Check sheet for the modelled part. Datum: model origin and axes. Units: mm. Face numbers are marked on the shaded views. Round coordinates to 2 decimals unless told otherwise and drop trailing zeros. Order: outer loops, then holes, each group sorted by start corner. A loop starts at its lowest first (then second) coordinate and runs counter-clockwise, first axis right, second up. Notation, with made-up numbers: (54.25, 58.25) -> (112.25, 58.25) arc R9 cw to (112.25, 69.25) -> close; hole circle Ø10 at (52.5, 29). An arc over 180 degrees is marked (long way). Answer in a Markdown table with one row per item.
from build123d import *

# Parameters (mm, degrees)
EXTRUDE_1_DEPTH             = 1.5
SKETCH_2_W                  = 12.5
SKETCH_2_H                  = 13.5
HOLE_WIZARD_12_0_12_1_D     = 12
HOLE_WIZARD_12_0_12_1_DEPTH = 13.5
SKETCH_5_W                  = 1.65
SKETCH_5_H                  = 11.731334643
HOLE_WIZARD_3_3_3_3_2_D     = 3.3
HOLE_WIZARD_3_3_3_3_2_DEPTH = 41.731334643
FILLET_1_R                  = 3


with BuildPart() as part:
    # 草图1 → 凸台-拉伸1 (new body)
    with BuildSketch(Plane.XY.offset(0.75)):
        with BuildLine():
            Line((17.5, 6), (47.11952886, 6))
            ThreePointArc((47.11952886, 6), (0, 47.5), (-47.11952886, 6))
            Line((-47.11952886, 6), (-17.5, 6))
            Line((-17.5, 6), (-17.5, 0))
            ThreePointArc((-17.5, 0), (0, -17.5), (17.5, 0))
            Line((17.5, 0), (17.5, 6))
        make_face()
    extrude(amount=-EXTRUDE_1_DEPTH)

    # 草图2 → 旋转1 (revolve)
    with BuildSketch(Plane(origin=(0, 0, 0), x_dir=(1, 0, 0), z_dir=(0, 1, 0))):
        with Locations((6.25, 7.5)):
            Rectangle(SKETCH_2_W, SKETCH_2_H)
    revolve(axis=Axis((0, 0, -14.25), (0, 0, 1)))

    # Ø12.0 (12) 直径孔1
    with Locations(Plane(origin=(0, 0, -14.25), x_dir=(-1, 0, 0), z_dir=(0, 0, -1))):
        with Locations((0, 0)):
            Hole(HOLE_WIZARD_12_0_12_1_D / 2, depth=HOLE_WIZARD_12_0_12_1_DEPTH)

    # 草图5 → Ø3.3 (3.3) 直径孔1 (revolve, cut)
    with BuildSketch(Plane(origin=(0, -5.768665357, -9.25), x_dir=(0, 0, 1), z_dir=(1, 0, 0))):
        with Locations((0.825, 5.865667322)):
            Rectangle(SKETCH_5_W, SKETCH_5_H)
    revolve(axis=Axis((0, 0.581334643, -9.25), (0, -1, 0)), mode=Mode.SUBTRACT)

    # Ø3.3 (3.3) 直径孔2
    with Locations(Plane(origin=(0, 5.768665357, 0), x_dir=(-1, 0, 0), z_dir=(0, -1, 0))):
        with Locations((0, 9.25)):
            Hole(HOLE_WIZARD_3_3_3_3_2_D / 2, depth=HOLE_WIZARD_3_3_3_3_2_DEPTH)

    # 圆角1
    fillet_1_edges = [part.edges().sort_by_distance(p)[0] for p in [
        (-17.5, 6, 0),
        (-47.11952886, 6, 0),
        (47.11952886, 6, 0),
        (17.5, 6, 0),
    ]]
    fillet(fillet_1_edges, radius=FILLET_1_R)


solid = part.part
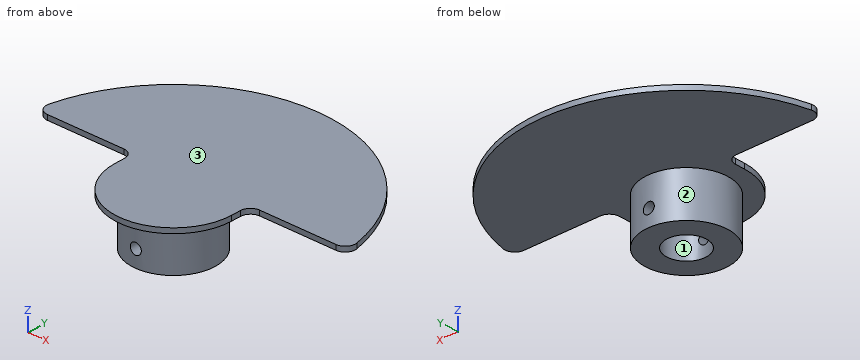
Item 1: Cross-section at B-B (z = -9.25). Record the boundary of the cut face in (x, y), and give its area (3 significant figures).
Result sheet:
| item | result |
|---|---|
| outline | (-1.65, -12.39) -> (-1.65, -5.77) arc R6 cw to (-1.65, 5.77) -> (-1.65, 12.39) arc R12.5 ccw to start; (1.65, -12.39) arc R12.5 ccw to (1.65, 12.39) -> (1.65, 5.77) arc R6 cw to (1.65, -5.77) -> close |
| area | 335 mm^2 |
Item 2: Cross-section at A-A (x = 0). Record the boundary of the cut face in (y, z).
Result sheet:
| item | result |
|---|---|
| outline | (-17.5, -0.75) -> (-12.5, -0.75) -> (-12.5, -7.6) -> (-6, -7.6) -> (-6, -0.75) -> (6, -0.75) -> (6, -7.6) -> (12.5, -7.6) -> (12.5, -0.75) -> (47.5, -0.75) -> (47.5, 0.75) -> (-17.5, 0.75) -> close; (-12.5, -14.25) -> (-6, -14.25) -> (-6, -10.9) -> (-12.5, -10.9) -> close; (6, -14.25) -> (12.5, -14.25) -> (12.5, -10.9) -> (6, -10.9) -> close |
Item 3: Depth check by flat-ended pin: P1, Ø1.2, axis at y = 2, z = 0.5, coming from the +X side; P2, Ø8, axis at y = -8.5, z = -6, coming from the -X side; P3, Ø0.8, axis at y = 1, z = 0, coming from the -X side; P4, Ø19, axis at x = 0, y = 0, coming from the -Z side. Enter the tip coordinate at first touch or a pass-through.
Result sheet:
| item | result |
|---|---|
| P1 | stops at x = 17.5 |
| P2 | stops at x = -11.66 |
| P3 | stops at x = -17.5 |
| P4 | stops at z = -14.25 |
Item 4: Mould release check, pull along Y, two halves, no side actions. Record for the marked faces 1, 2 and 3: pulls with the +Y half, pulls with the -Y half, needs draft (parallel to the pull), parting line crosses it, or undercut.
Result sheet:
| item | result |
|---|---|
| face 1 | undercut |
| face 2 | parting line crosses it |
| face 3 | needs draft |
Item 5: Scan lines: line 1 (Y direction, x = 0, z = -4); line 2 (Z direction, x = 0, y = -9); line 3 (Z direction, x = -27, y = 23.5). Record each from-to range of solid material in increasing order. Write a range as [from, to].
Result sheet:
| item | result |
|---|---|
| line 1 | y = [-12.5, -6], [6, 12.5] |
| line 2 | z = [-14.25, -10.9], [-7.6, 0.75] |
| line 3 | z = [-0.75, 0.75] |
Item 6: Cross-section at D-D (x = -14.5). Record the boundary of the cut face in (y, z).
Result sheet:
| item | result |
|---|---|
| outline | (-9.8, -0.75) -> (45.23, -0.75) -> (45.23, 0.75) -> (-9.8, 0.75) -> close |
Item 7: Cross-section at C-C (y = -4). Record the boundary of the cut face in (x, z).
Result sheet:
| item | result |
|---|---|
| outline | (-17.04, -0.75) -> (-11.84, -0.75) -> (-11.84, -14.25) -> (-4.47, -14.25) -> (-4.47, -0.75) -> (4.47, -0.75) -> (4.47, -14.25) -> (11.84, -14.25) -> (11.84, -0.75) -> (17.04, -0.75) -> (17.04, 0.75) -> (-17.04, 0.75) -> close |
